The model under review builds one solid part; all positions refer to its coordinate system, in mm. Round coordinates to 2 decimals unless told otherwise and drop trailing zeros. Loops run counter-clockwise (first coordinate to the right, second up) from the corner with the lowest first, then second, coordinate; pieces in that order, holes last. Notation, with made-up numbers: (40.5, 55) -> (73.5, 55) arc R31 ccw to (73.5, 85) -> close; hole circle Ø3 at (65, -32). An arc over 180 degrees is marked (long way). Use a Markdown table: item, result. Add a question column.
1) Consider section A-A on y = 1081. Give the boundary of the cut face in (x, z).
2) Consider section C-C on z = 1.15. Give the boundary of the cut face in (x, y).
3) Insertion check: pin 1 (2 mm diameter, centred on y = 1770, z = 4, fed in from -X). The pin has a flat end and moves straight along its axis. Give the tip position at first contact, or say it passes through.
4) Wall thickness on probe 1 along Y at (x, z) = (601.5, 0.4); probe 2 along X at (y, z) = (1796, 2.4): over which ranges is each line inside the solid? List them lowest first.
5) Consider section B-B on x = 606.5. Give the boundary of the cut face in (y, z), plus the area to 3 significant figures.
from build123d import *

# Parameters (mm, degrees)
SKETCH1_W           = 1110.611762236
SKETCH1_H           = 2124
SKETCH1_W_2         = 805.022462921
SKETCH1_H_2         = 275.761568038
BOSS_EXTRUDE1_DEPTH = 5


with BuildPart() as part:
    # Sketch1 → Boss-Extrude1 (new body)
    with BuildSketch(Plane.XY):
        with Locations((555.305881118, 1062)):
            Rectangle(SKETCH1_W, SKETCH1_H)
        with Locations((609.562824722, 1925.776054905)):
            Rectangle(SKETCH1_W_2, SKETCH1_H_2, mode=Mode.SUBTRACT)
        with Locations((609.562824722, 1068.55899332)):
            Rectangle(SKETCH1_W_2, SKETCH1_H_2, mode=Mode.SUBTRACT)
        with Locations((609.562824722, 198.131798559)):
            Rectangle(SKETCH1_W_2, SKETCH1_H_2, mode=Mode.SUBTRACT)
    extrude(amount=BOSS_EXTRUDE1_DEPTH)


solid = part.part
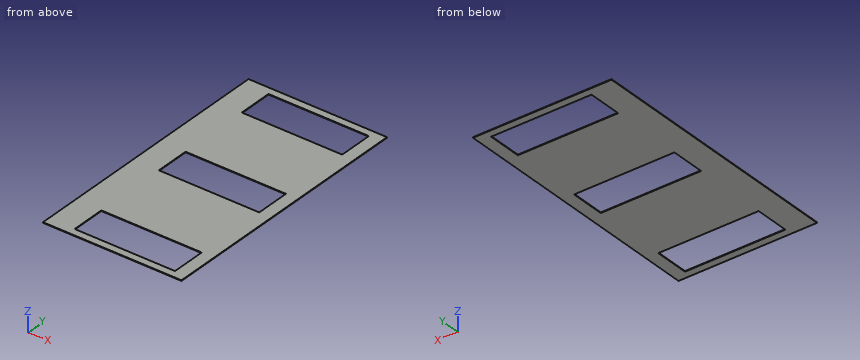
Result set:
| question | item | result |
|---|---|---|
| 1 | outline | (0, 0) -> (207.05, 0) -> (207.05, 5) -> (0, 5) -> close; (1012.07, 0) -> (1110.61, 0) -> (1110.61, 5) -> (1012.07, 5) -> close |
| 2 | outline | (0, 0) -> (1110.61, 0) -> (1110.61, 2124) -> (0, 2124) -> close; hole (207.05, 60.25) -> (1012.07, 60.25) -> (1012.07, 336.01) -> (207.05, 336.01) -> close; hole (207.05, 930.68) -> (1012.07, 930.68) -> (1012.07, 1206.44) -> (207.05, 1206.44) -> close; hole (207.05, 1787.9) -> (1012.07, 1787.9) -> (1012.07, 2063.66) -> (207.05, 2063.66) -> close |
| 3 | pin 1 | x = 0 |
| 4 | probe 1 | 0 to 60.25, 336.01 to 930.68, 1206.44 to 1787.9, 2063.66 to 2124 |
| 4 | probe 2 | 0 to 207.05, 1012.07 to 1110.61 |
| 5 | outline | (0, 0) -> (60.25, 0) -> (60.25, 5) -> (0, 5) -> close; (336.01, 0) -> (930.68, 0) -> (930.68, 5) -> (336.01, 5) -> close; (1206.44, 0) -> (1787.9, 0) -> (1787.9, 5) -> (1206.44, 5) -> close; (2063.66, 0) -> (2124, 0) -> (2124, 5) -> (2063.66, 5) -> close |
| 5 | area | 6,480 mm2 |
